from build123d import *

# Parameters (mm, degrees)
PLATE_PROFILE_SKETCH_R    = 22.5
BASE_PLATE_65X50X3_DEPTH  = 3
CENTRE_HOLE_SKETCH_R      = 7.306731966
CENTRE_THROUGH_HOLE_DEPTH = 3


with BuildPart() as part:
    # Plate Profile Sketch → Base Plate 65x50x3 (new body)
    with BuildSketch(Plane.XY):
        with BuildLine():
            Line((-26.5, -25), (26.5, -25))
            ThreePointArc((26.5, -25), (30.742640687, -23.242640687), (32.5, -19))
            Line((32.5, -19), (32.5, 19))
            ThreePointArc((32.5, 19), (30.742640687, 23.242640687), (26.5, 25))
            Line((26.5, 25), (-26.5, 25))
            ThreePointArc((-26.5, 25), (-30.742640687, 23.242640687), (-32.5, 19))
            Line((-32.5, 19), (-32.5, -19))
            ThreePointArc((-32.5, -19), (-30.742640687, -23.242640687), (-26.5, -25))
        make_face()
        Circle(PLATE_PROFILE_SKETCH_R, mode=Mode.SUBTRACT)
    extrude(amount=BASE_PLATE_65X50X3_DEPTH)

    # Conical Dimple Profile Sketch → Conical Dimple (revolve)
    with BuildSketch(Plane(origin=(0, 0, 0), x_dir=(1, 0, 0), z_dir=(0, 1, 0))):
        with BuildLine():
            Line((13.091820453, 7.894399988), (20.827095747, 1.403733341))
            ThreePointArc((20.827095747, 1.403733341), (22.631700546, 0.361844275), (24.683821406, 0))
            Line((24.683821406, 0), (20.16641426, 0))
            Line((20.16641426, 0), (12.127639038, 6.745333323))
            ThreePointArc((12.127639038, 6.745333323), (9.871883041, 8.047694656), (7.306731966, 8.5))
            Line((7.306731966, 8.5), (0, 8.5))
            Line((0, 8.5), (0, 10))
            Line((0, 10), (7.306731966, 10))
            ThreePointArc((7.306731966, 10), (10.384913256, 9.457233587), (13.091820453, 7.894399988))
        make_face()
    revolve(axis=Axis((0, 0, 5.787775716), (0, 0, -1)))

    # Centre Hole Sketch → Centre Through Hole (cut)
    with BuildSketch(Plane(origin=(0, 0, -10), x_dir=(-1, 0, 0), z_dir=(0, 0, -1))):
        with Locations(Location((0, 0, 0), (0, 0, 180))):
            Circle(CENTRE_HOLE_SKETCH_R)
    extrude(amount=-CENTRE_THROUGH_HOLE_DEPTH, mode=Mode.SUBTRACT)


solid = part.part
Source: CAD feature listing. Evaluate the final solid. Frame: model axes, mm. A direction names the side the tool comes from. Coordinates: 2 decimals unless noted, no trailing zeros. Loops run counter-clockwise (first coordinate to the right, second up) from the corner with the lowest first, then second, coordinate; pieces in that order, holes last. Notation, with made-up numbers: (69.5, -19) - (103.5, -19) arc R9 cw to (103.5, -2) - close; hole circle Ø4 at (61.25, -21.75). An arc over 180 degrees is marked (long way). Return JSON: item names as keys, results as strings.
Q1. Section A-A, the plane z = 1.75. Return loops of the section in (x, y).
Results:
{"outline": "(-32.5, -19) arc R6 ccw to (-26.5, -25) - (26.5, -25) arc R6 ccw to (32.5, -19) - (32.5, 19) arc R6 ccw to (26.5, 25) - (-26.5, 25) arc R6 ccw to (-32.5, 19) - close; hole circle Ø45 at (0, 0)"}
Q2. Material intervals for line 1 along Y through (x, z) = (0, 0.8); line 2 along X through (y, z) = (-2, -0.5); line 3 along X through (y, z) = (0, -9), sorted ascending.
Results:
{"line 1": "-25 to -22.5, 22.5 to 25", "line 2": "-22.2 to -19.47, 19.47 to 22.2", "line 3": "-11.43 to -7.31, 7.31 to 11.43"}
Q3. Mould query, pull axis Y, two halves, no side actions, for faces 4 (the cylindrical face through (30.789, 23.196, 1.479)), 5 (the conical face through (-2.71, 12.22, -6.42)), 6 (the conical face through (12.949, -4.078, -7.488)). Classes: released by +Y, released by -Y, zero draft, split by the parting line, or undercut.
Results:
{"face 4": "released by +Y", "face 5": "undercut", "face 6": "split by the parting line"}
Q4. Contact query for flat-ended pins moving along their axis: P1, Ø4, axis at y = 1.5, z = -4.5, coming from the +X side; P2, Ø1, axis at x = -7.5, z = -4.5, coming from the +Y side; P3, Ø22.5, axis at x = 0, y = 8, coming from the +Z side; P4, Ø13, axis at x = 0, y = 0, coming from the +Z side. Output: stop coordinate, or through.
Results:
{"P1": "x = 19.47", "P2": "y = 16.11", "P3": "z = -0.77", "P4": "through"}
Q5. Access query for faces 1 (the cylindrical face through (10.382, -19.961, 1.479)), 2 (the flat face through (0, -25, 1)), 3 (the flat face through (-22.1, 11.5, 0)). Directions: +Z, -Z, +X, -X, +Y, -Y. A direction counts if a zero-diameter tool reaches every point of the face in a straight line with its end or side. Return the directions, or none.
Results:
{"face 1": "+Z", "face 2": "+Z, -Z, +X, -X, -Y", "face 3": "-Z"}
